from build123d import *

# Parameters (mm, degrees)
BOSS_EXTRUDE1_DEPTH   = 8
M5_TAPPED_HOLE1_D     = 4.2
M5_TAPPED_HOLE1_DEPTH = 12.4
M5_TAPPED_HOLE1_TIP   = 1.2618073
M4_TAPPED_HOLE1_D     = 3.3
M4_TAPPED_HOLE1_DEPTH = 10.1
M4_TAPPED_HOLE1_TIP   = 0.991420021


with BuildPart() as part:
    # Sketch1 → Boss-Extrude1 (new body)
    with BuildSketch(Plane.XY):
        with BuildLine():
            Line((-45, 50), (45, 50))
            ThreePointArc((45, 50), (48.535533906, 48.535533906), (50, 45))
            Line((50, 45), (50, -45))
            ThreePointArc((50, -45), (48.535533906, -48.535533906), (45, -50))
            Line((45, -50), (-45, -50))
            ThreePointArc((-45, -50), (-48.535533906, -48.535533906), (-50, -45))
            Line((-50, -45), (-50, 45))
            ThreePointArc((-50, 45), (-48.535533906, 48.535533906), (-45, 50))
        make_face()
    extrude(amount=BOSS_EXTRUDE1_DEPTH)

    # M5 Tapped Hole1
    with Locations(Plane(origin=(-43, 43, 8), x_dir=(1, 0, 0), z_dir=(0, 0, 1))):
        with Locations((0, 0), (86, 0), (86, -86), (0, -86)):
            Hole(M5_TAPPED_HOLE1_D / 2, depth=M5_TAPPED_HOLE1_DEPTH)
            with Locations((0, 0, -(M5_TAPPED_HOLE1_DEPTH + M5_TAPPED_HOLE1_TIP / 2))):  # 118° drill point
                Cone(0, M5_TAPPED_HOLE1_D / 2, M5_TAPPED_HOLE1_TIP, mode=Mode.SUBTRACT)

    # M4 Tapped Hole1
    with Locations(Plane(origin=(-30, -45, 8), x_dir=(1, 0, 0), z_dir=(0, 0, 1))):
        with Locations((0, 0), (60, 0), (-15, 15), (-15, 75), (75, 75), (75, 15), (0, 90), (60, 90)):
            Hole(M4_TAPPED_HOLE1_D / 2, depth=M4_TAPPED_HOLE1_DEPTH)
            with Locations((0, 0, -(M4_TAPPED_HOLE1_DEPTH + M4_TAPPED_HOLE1_TIP / 2))):  # 118° drill point
                Cone(0, M4_TAPPED_HOLE1_D / 2, M4_TAPPED_HOLE1_TIP, mode=Mode.SUBTRACT)


solid = part.part
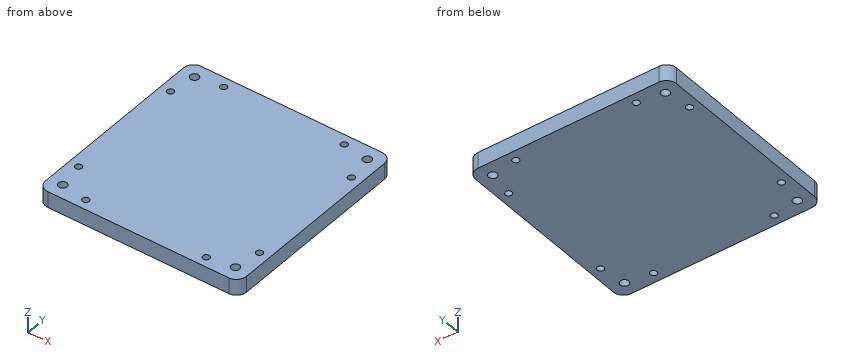
Work out the finished part from the listing and answer in its coordinate system (mm). Round coordinates to 2 decimals unless told otherwise and drop trailing zeros. Write each loop counter-clockwise with the first axis right and the second up, starting at its lowest first coordinate (ties: lowest second). Pieces come first, ordered by that corner, then holes. Notation, with made-up numbers: (52, 78) - (57, 78) arc R27 ccw to (57, 97) - close; hole circle Ø5 at (30.25, 57). An arc over 180 degrees is marked (long way). Answer in a Markdown table with one row per item. Add a question column.
1. A cutting plane is placed at A-A, the plane y = 30. Determine the outline of the cut face in (x, z).
2. Given pin 1 (2.5 mm diameter, centred on x = -30, y = -45, fed in from +Z), flat-ended and moving along its own axis, determine where the tip first touches the part or whether it passes through.
3. Find the intervals of material crossed by line 1 along Y through (x, z) = (-30, 3); line 2 along Y through (x, z) = (43, 2), in increasing order. Write a range as from..to.
Worked out:
| question | item | result |
|---|---|---|
| 1 | outline | (-50, 0) - (-46.65, 0) - (-46.65, 8) - (-50, 8) - close; (-43.35, 0) - (43.35, 0) - (43.35, 8) - (-43.35, 8) - close; (46.65, 0) - (50, 0) - (50, 8) - (46.65, 8) - close |
| 2 | pin 1 | through |
| 3 | line 1 | -50..-46.65, -43.35..43.35, 46.65..50 |
| 3 | line 2 | -50..-45.1, -40.9..40.9, 45.1..50 |
